Read the model definition and answer for the solid it produces. Units are mm, in the model's axes. Face numbers are marked on the shaded views. A direction names the side the tool comes from. Round coordinates to 2 decimals unless told otherwise and drop trailing zeros. Loops run counter-clockwise (first coordinate to the right, second up) from the corner with the lowest first, then second, coordinate; pieces in that order, holes last. Notation, with made-up numbers: (38, -18) - (76, -18) arc R24 ccw to (76, 10) - close; hole circle Ø6 at (-9.75, 22). An arc over 180 degrees is marked (long way). Use CSV: the item, a comma, the result in double quotes. Start each with the question number.
1. Find section D-D (x = 52). Give the vertices of the cut face in (y, z), and give its area (3 significant figures).
2. Find section B-B (y = 48). Give the vertices of the cut face in (x, z), and give its area (3 significant figures).
3. Find section C-C (z = 30). Give the vertices of the cut face in (x, y), and give its area (3 significant figures).
4. Consider line 1 along X through (y, z) = (35, 27); line 2 along Y through (x, z) = (70, 43); line 3 along Y through (x, z) = (10, 27.5). Determine where each line is inside the solid, lowest interval first.
5. A tool of negligible diameter and unlimited length cuts with its end or side. For the marked faces 4, 5, 6 and 7, from which of +Z, -Z, +X, -X, +Y, -Y can it reach the whole face along a straight path? Write none if from no direction.
6. Find section A-A (z = 6). Give the vertices of the cut face in (x, y).
7. Given pin 1 Ø8 at (x, z) = (59, 20) entering from +Y; pin 2 Ø6 at (x, y) = (11.5, 32.5) entering from +Z; pin 3 Ø4 at (y, z) = (27, 18) entering from -X; pin 4 Ø6 at (x, z) = (87.5, 15.5) entering from +Y, each flat-ended and moving along its own axis, determine where each tip first touches the part or whether it passes through.
8. Determine the mould class of the marked faces 1, 2 and 3 for opening direction Z: +Z half, -Z half, draft (parallel to the pull), parting line (faces both ways), or undercut.
from build123d import *

# Parameters (mm, degrees)
BLOCK_BODY_DEPTH          = 50
BEARING_START             = -13
BEARING_ARC_RECESS_DEPTH  = 13
ARC_POCKET_SKETCH_R       = 10.03476875
ARC_POCKET_SKETCH_R_2     = 5
ARC_POCKET_DEPTH          = 8
PIN_10_SKETCH_R           = 5
PIN_10_DEPTH              = 8
SIDE_BOSS_DEPTH           = 8
PROFILE_RELIEF_CUT_DEPTH  = 129.33160172
STEP_CUT_DEPTH            = 9
STEP_NOTCH_DEPTH          = 126.099960032
SLOT_CUT_SKETCH_R         = 5
SLOT_CUT_DEPTH            = 129.33160172
TOP_RELIEF_CUT_DEPTH      = 129.33160172
TOP_RELIEF_CUT_DEPTH_BACK = 129.33160172
TOP_RELIEF_SKETCH_W       = 10
TOP_RELIEF_SKETCH_H       = 12


with BuildPart() as part:
    # Block Profile Sketch → Block Body (new body)
    with BuildSketch(Plane.XY):
        with BuildLine():
            ThreePointArc((70, 35), (78.786796564, 13.786796564), (100, 5))
            Line((100, 5), (100, 0))
            Line((100, 0), (0, 0))
            Line((0, 0), (0, 53))
            Line((0, 53), (40, 53))
            Line((40, 53), (40, 63))
            Line((40, 63), (50, 63))
            Line((50, 63), (68, 63))
            Line((68, 63), (70, 53))
            Line((70, 53), (70, 35))
        make_face()
    extrude(amount=BLOCK_BODY_DEPTH)

    # Bearing Arc Recess Sketch → Bearing Arc Recess (cut)
    with BuildSketch(Plane.XY.offset(50).offset(BEARING_START)):
        with BuildLine():
            ThreePointArc((80.416666667, 12.273516428), (91.040635288, 21.498456878), (95, 35))
            ThreePointArc((95, 35), (87.17838735, 53.163232313), (68.607759357, 59.961203216))
            Line((68.607759357, 59.961203216), (70, 53))
            Line((70, 53), (70, 45))
            ThreePointArc((70, 45), (77.071067812, 42.071067812), (80, 35))
            ThreePointArc((80, 35), (77.637626158, 28.545027756), (71.666666667, 25.139867028))
            ThreePointArc((71.666666667, 25.139867028), (75.192995333, 18.129537071), (80.416666667, 12.273516428))
        make_face()
        with BuildLine():
            Line((70, 53), (68.607759357, 59.961203216))
            ThreePointArc((68.607759357, 59.961203216), (45.732966105, 28.990751633), (80.416666667, 12.273516428))
            ThreePointArc((80.416666667, 12.273516428), (75.192995333, 18.129537071), (71.666666667, 25.139867028))
            ThreePointArc((71.666666667, 25.139867028), (60.035028105, 34.163737397), (70, 45))
            Line((70, 45), (70, 53))
        make_face()
    extrude(amount=BEARING_ARC_RECESS_DEPTH, mode=Mode.SUBTRACT)

    # Arc Pocket Sketch → Arc Pocket (cut)
    with BuildSketch(Plane.XY.offset(50)):
        with Locations((70, 35)):
            Circle(ARC_POCKET_SKETCH_R)
        with Locations((70, 35)):
            Circle(ARC_POCKET_SKETCH_R_2, mode=Mode.SUBTRACT)
    extrude(amount=-ARC_POCKET_DEPTH, mode=Mode.SUBTRACT)

    # Pin _10 Sketch → Pin _10 (add)
    with BuildSketch(Plane.XY.offset(50)):
        with Locations((70, 35)):
            Circle(PIN_10_SKETCH_R)
    extrude(amount=-PIN_10_DEPTH)

    # Side Boss Sketch → Side Boss (add)
    with BuildSketch(Plane.XY.offset(50)):
        with BuildLine():
            Line((80.416666667, 12.273516428), (80.416666667, 0))
            Line((80.416666667, 0), (100, 0))
            Line((100, 0), (100, 8))
            ThreePointArc((100, 8), (89.761290268, 8.088189193), (80.416666667, 12.273516428))
        make_face()
    extrude(amount=-SIDE_BOSS_DEPTH)

    # Profile Relief Sketch → Profile Relief Cut (cut, through all)
    with BuildSketch(Plane.XY.offset(50)):
        with BuildLine():
            Line((20.629839756, 5.629839756), (15, 0))
            Line((15, 0), (25, 0))
            Line((25, 0), (55, 0))
            Line((55, 0), (30.863185228, 8.045604924))
            ThreePointArc((30.863185228, 8.045604924), (25.403378362, 8.291261838), (20.629839756, 5.629839756))
        make_face()
    extrude(amount=-PROFILE_RELIEF_CUT_DEPTH, mode=Mode.SUBTRACT)

    # Step Cut Sketch → Step Cut (cut)
    with BuildSketch(Plane.XY.offset(50)):
        with BuildLine():
            Line((0, 35), (20, 35))
            ThreePointArc((20, 35), (16.946326412, 45.621771092), (8.717797887, 53))
            Line((8.717797887, 53), (0, 53))
            Line((0, 53), (0, 35))
        make_face()
        with BuildLine():
            ThreePointArc((8.717797887, 53), (16.946326412, 45.621771092), (20, 35))
            Line((20, 35), (20, 53))
            Line((20, 53), (8.717797887, 53))
        make_face()
        with BuildLine():
            ThreePointArc((0, 15), (14.142135624, 20.857864376), (20, 35))
            Line((20, 35), (0, 35))
            Line((0, 35), (0, 15))
        make_face()
    extrude(amount=-STEP_CUT_DEPTH, mode=Mode.SUBTRACT)

    # Step Notch Sketch → Step Notch (cut, through all)
    with BuildSketch(Plane.XY.offset(41)):
        with BuildLine():
            ThreePointArc((10, 40), (6.464466094, 31.464466094), (15, 35))
            Line((15, 35), (10, 35))
            Line((10, 35), (10, 40))
        make_face()
        with BuildLine():
            Line((10, 35), (15, 35))
            ThreePointArc((15, 35), (13.535533906, 38.535533906), (10, 40))
            Line((10, 40), (10, 35))
        make_face()
    extrude(amount=-STEP_NOTCH_DEPTH, mode=Mode.SUBTRACT)

    # Slot Cut Sketch → Slot Cut (cut, through all)
    with BuildSketch(Plane(origin=(0, 63, 0), x_dir=(1, 0, 0), z_dir=(0, 1, 0))):
        with Locations(Location((59, -20, 0), (0, 0, 270))):
            Circle(SLOT_CUT_SKETCH_R)
    extrude(amount=-SLOT_CUT_DEPTH, mode=Mode.SUBTRACT)

    # Top Relief Sketch → Top Relief Cut (cut, two sides: drawn at the far end of the back side and taken through both)
    with BuildSketch(Plane(origin=(0, 63, 0), x_dir=(1, 0, 0), z_dir=(0, 1, 0)).offset(-TOP_RELIEF_CUT_DEPTH_BACK)):
        with Locations((45, -6)):
            Rectangle(TOP_RELIEF_SKETCH_W, TOP_RELIEF_SKETCH_H)
        Polygon((40, -12), (40, 0), (0, 0), (0, -20.5), (40, -20.161016949), align=None)
    extrude(amount=TOP_RELIEF_CUT_DEPTH + TOP_RELIEF_CUT_DEPTH_BACK, mode=Mode.SUBTRACT)


solid = part.part
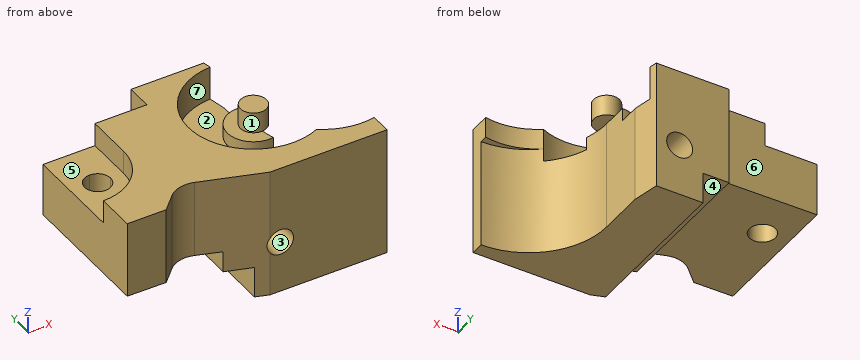
Filled sheet:
1,outline,"(1, 0) - (63, 0) - (63, 50) - (52.35, 50) - (52.35, 37) - (17.65, 37) - (17.65, 50) - (1, 50) - close"
1,area,"2,650 mm²"
2,outline,"(0, 20.5) - (40, 20.16) - (40, 12) - (50, 12) - (50, 0) - (70, 0) - (70, 37) - (48.65, 37) - (48.65, 50) - (20, 50) - (20, 41) - (0, 41) - close; hole circle Ø10 at (59, 20)"
2,area,"2,030 mm²"
3,outline,"(0, 0) - (15, 0) - (20.63, 5.63) arc R10 cw to (30.86, 8.05) - (55, 0) - (100, 0) - (100, 5) arc R30 cw to (70, 35) - (70, 53) - (68, 63) - (40, 63) - (40, 53) - (0, 53) - close; hole circle Ø10 at (10, 35)"
3,area,"4,070 mm²"
4,line 1,"x = 0 to 5, 15 to 70"
4,line 2,"y = 0 to 10, 30 to 40"
4,line 3,"y = 0 to 30, 40 to 53"
5,face 4,"-Z, -X, +Y, -Y"
5,face 5,"+Z, -X, +Y"
5,face 6,"+Z, -Z, -X, +Y"
5,face 7,"+Z"
6,outline,"(50, 1.67) - (55, 0) - (100, 0) - (100, 5) arc R30 cw to (70, 35) - (70, 53) - (68, 63) - (50, 63) - close"
7,pin 1,"passes through"
7,pin 2,"stops at z = 41"
7,pin 3,"stops at x = 40"
7,pin 4,"stops at y = 9.31"
8,face 1,"draft"
8,face 2,"+Z half"
8,face 3,"undercut"
